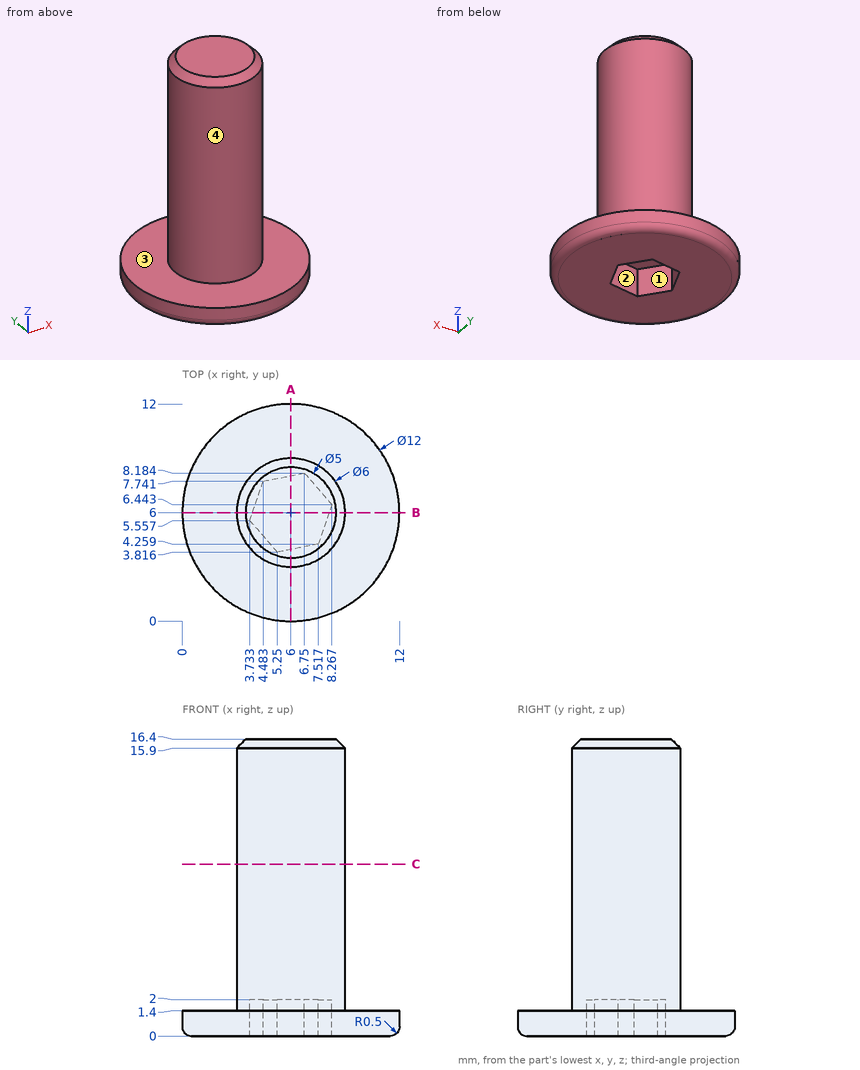
Here's the drawing with two shaded views (mm, measured from the low corner). I have some questions. Give positions to 0.01 mm unless a question says otherwise; leave off trailing zeros. Order: outer loops, then holes, each group sorted by start corner. A loop starts at its lowest first (then second) coordinate and runs counter-clockwise, first axis right, second up. Notation, with made-up numbers: (60.5, 37.25) -> (73.5, 37.25) arc R11 ccw to (73.5, 52.25) -> close; hole circle Ø11 at (21.5, 68). An arc over 180 degrees is marked (long way). One line per item, written item: value. Start each with the question number.
1. Will these pins go through, and if not, where does the flat tip stop? pin 1 Ø3 at (x, y) = (1.5, 5) entering from +Z; pin 2 Ø4 at (y, z) = (4, 13) entering from -X; pin 3 Ø3 at (x, z) = (6.5, 4) entering from -Y.
2. Imagine slicing it at B-B, the plane y = 6. List the corners of the cut face in (x, z) for me (1 decimal).
3. We'd pull the mould along X, two halves only. Please class the marked faces 1, 2, 3 and 4: released by +X, released by -X, zero draft, split by the parting line, or undercut.
4. Imagine slicing it at A-A, the plane x = 6. List the corners of the cut face in (y, z) for me.
5. I need wall thicknesses on probe 1 along Z at (x, y) = (7.5, 10); probe 2 along Z at (x, y) = (5.25, 5.5); probe 3 along Y at (x, z) = (5.25, 8.75) (1 decimal). Which ranges of each line are inside material? Lowest first, please. Write a range as from..to.
6. Imagine slicing it at C-C, the plane z = 9.5. List the corners of the cut face in (x, y) for me, plus the area to 3 significant figures.
Values follow:
1. pin 1: stops at z = 1.4
1. pin 2: stops at x = 3
1. pin 3: stops at y = 3
2. outline: (0, 0.5) arc R0.5 ccw to (0.5, 0) -> (3.9, 0) -> (3.9, 2) -> (8.1, 2) -> (8.1, 0) -> (11.5, 0) arc R0.5 ccw to (12, 0.5) -> (12, 1.4) -> (9, 1.4) -> (9, 15.9) -> (8.5, 16.4) -> (3.5, 16.4) -> (3, 15.9) -> (3, 1.4) -> (0, 1.4) -> close
3. face 1: undercut
3. face 2: undercut
3. face 3: zero draft
3. face 4: split by the parting line
4. outline: (0, 0.5) arc R0.5 ccw to (0.5, 0) -> (3.96, 0) -> (3.96, 2) -> (8.04, 2) -> (8.04, 0) -> (11.5, 0) arc R0.5 ccw to (12, 0.5) -> (12, 1.4) -> (9, 1.4) -> (9, 15.9) -> (8.5, 16.4) -> (3.5, 16.4) -> (3, 15.9) -> (3, 1.4) -> (0, 1.4) -> close
5. probe 1: z = 0..1.4
5. probe 2: z = 2..16.4
5. probe 3: y = 3.1..8.9
6. outline: circle Ø6 at (6, 6)
6. area: 28.3 mm2
